```python
from build123d import *

# Parameters (mm, degrees)
SKETCH_1_R          = 17.5
EXTRUDE_1_DEPTH     = 628.7
CUT_EXTRUDE_START   = -40
SKETCH_3_R          = 17.5
SKETCH_3_R_2        = 15
CUT_EXTRUDE_1_DEPTH = 40
CUT_EXTRUDE_2_DEPTH = 4
CUT_EXTRUDE_START_2 = 31.9
SKETCH_5_R          = 15
SKETCH_5_R_2        = 14.5
CUT_EXTRUDE_3_DEPTH = 1.3


with BuildPart() as part:
    # 草图1 → 凸台-拉伸1 (new body)
    with BuildSketch(Plane(origin=(0, 0, 0), x_dir=(0, 0, -1), z_dir=(1, 0, 0))):
        with Locations(Location((0, 0, 0), (0, 0, 180))):
            Circle(SKETCH_1_R)
    extrude(amount=EXTRUDE_1_DEPTH)

    # 草图3 → 切除-拉伸1 (cut)
    with BuildSketch(Plane(origin=(628.7, 0, 0), x_dir=(0, 0, -1), z_dir=(1, 0, 0)).offset(CUT_EXTRUDE_START)):
        with Locations(Location((0, 0, 0), (0, 0, 180))):
            Circle(SKETCH_3_R)
        Circle(SKETCH_3_R_2, mode=Mode.SUBTRACT)
    extrude(amount=CUT_EXTRUDE_1_DEPTH, mode=Mode.SUBTRACT)

    # 草图4 → 切除-拉伸2 (cut)
    with BuildSketch(Plane(origin=(0, 15, 0), x_dir=(1, 0, 0), z_dir=(0, 1, 0))):
        with BuildLine():
            Line((598.7, 4), (628.7, 4))
            Line((628.7, 4), (628.7, -4))
            Line((628.7, -4), (598.7, -4))
            ThreePointArc((598.7, -4), (594.7, 0), (598.7, 4))
        make_face()
    extrude(amount=-CUT_EXTRUDE_2_DEPTH, mode=Mode.SUBTRACT)

    # 草图5 → 切除-拉伸3 (cut)
    with BuildSketch(Plane(origin=(588.7, 0, 0), x_dir=(0, 0, -1), z_dir=(1, 0, 0)).offset(CUT_EXTRUDE_START_2)):
        Circle(SKETCH_5_R)
        Circle(SKETCH_5_R_2, mode=Mode.SUBTRACT)
    extrude(amount=CUT_EXTRUDE_3_DEPTH, mode=Mode.SUBTRACT)


solid = part.part
```
The listing builds one solid part. Answer for the finished solid, in the listing's coordinates (mm). A direction names the side the tool comes from. Give positions to 0.01 mm unless a question says otherwise; leave off trailing zeros. Order: outer loops, then holes, each group sorted by start corner. A loop starts at its lowest first (then second) coordinate and runs counter-clockwise, first axis right, second up. Notation, with made-up numbers: M -12,32.5 L 37,32.5 A12 ccw 37,44.5 Z; hole C 41.5,67.25 d11. An arc over 180 degrees is marked long. Put each result on its own line as item: value. Start each with the question number.
Item 1: Find the intervals of material crossed by line 1 along Y through (x, z) = (178.5, -1.5); line 2 along X through (y, z) = (13, 9); line 3 along Z through (x, y) = (75.5, -0.5), in increasing order.
Item 2: The part is cut by section A-A, the plane x = 286.5. Determine the outline of the cut face in (y, z).
Item 3: For a pull along X with two mould halves and no side action, classify faces 4 (the face through (0, 0, 0)), 5 (the face through (620.6, -2.4, 14.5)), 6 (the face through (628.7, 0, 0)) as +X half, -X half, draft (parallel to the pull), parting line (faces both ways), or undercut.
Item 4: Flat-ended cylindrical pins translate along their axes: P1, Ø1, axis at x = 343, y = -5, coming from the -Z side; P2, Ø2, axis at x = 509, y = -12, coming from the -Z side; P3, Ø1, axis at x = 614.5, y = 12, coming from the +Z side. Find the tip coordinate at first contact, or state that the pin passes through.
Item 5: Which of the six approach directions +Z, -Z, +X, -X, +Y, -Y give full straight-line access (tool end or side, diameter ignored) to faces 1 (the face through (290.229, 17.084, -3.794)), 2 (the face through (604.427, -14.643, 3.252)), 3 (the face through (621.24, -14.49, 0.58))?
Answer key:
1. line 1: y = -17.44 to 17.44
1. line 2: x = 0 to 588.7
1. line 3: z = -17.49 to 17.49
2. outline: C 0,0 d35
3. face 4: -X half
3. face 5: undercut
3. face 6: +X half
4. P1: stops at z = -16.91
4. P2: stops at z = -13.61
4. P3: stops at z = 9.63
5. face 1: +X, -X
5. face 2: +X
5. face 3: none
